Design review of the part shown in the three views and the two pictorial views. Dimensions are in mm from the part's minimum x, y and z. A direction names the side the tool comes from. Give positions to 0.01 mm unless a question says otherwise; leave off trailing zeros. Write each loop counter-clockwise with the first axis right and the second up, starting at its lowest first coordinate (ties: lowest second). Pieces come first, ordered by that corner, then holes. Notation, with made-up numbers: M 39.25,87.5 L 85.25,87.5 A23 ccw 85.25,101.5 Z; hole C -12.5,76.5 d2. An arc over 180 degrees is marked long. Write item = value, one per line.
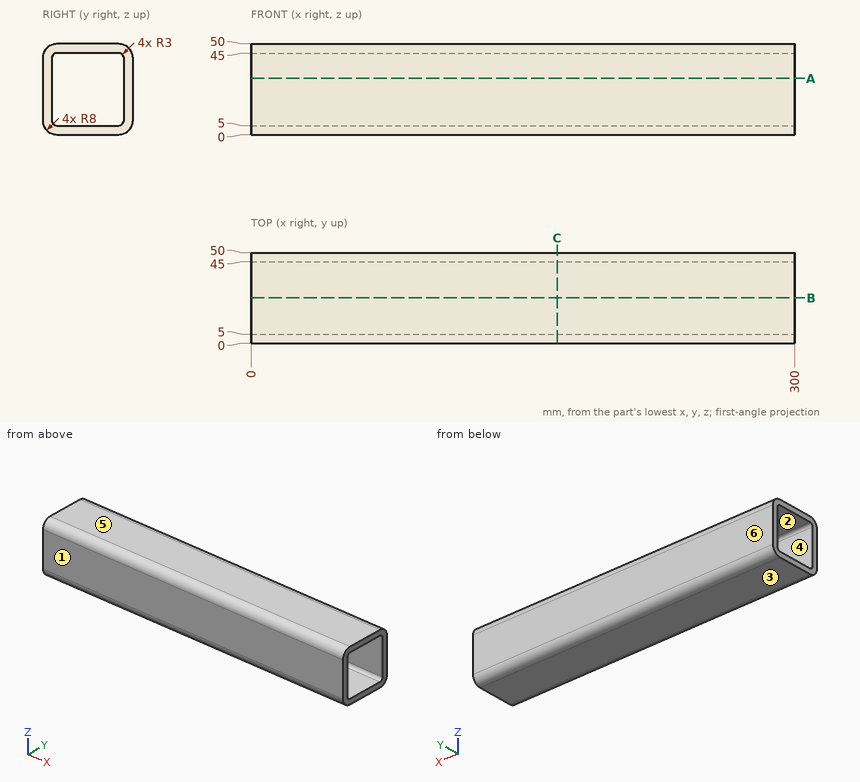
1. The part is to be moulded in two halves that separate along Z. For the marked faces 3, 4, 5 and 6, say which applies: +Z half, -Z half, draft (parallel to the pull), parting line (faces both ways), or undercut.
Responses:
face_3 = -Z half
face_4 = undercut
face_5 = +Z half
face_6 = draft
2. Insertion check: P1, Ø10, axis at y = 14, z = 39.5, coming from the -X side; P2, Ø4, axis at x = 216, y = 5.5, coming from the -Z side. Each pin has a flat end and moves straight along its axis. Give the tip position at first contact, or say it passes through.
Responses:
P1 = through
P2 = 0.02
3. We need section A-A, the plane z = 31. Write out the cut boundary in (x, y).
Responses:
outline = M 0,0 L 300,0 L 300,5 L 0,5 Z; M 0,45 L 300,45 L 300,50 L 0,50 Z
4. Machinability: for the marked faces 1 and 2, which of the approach directions +Z, -Z, +X, -X, +Y, -Y give a long, thin tool a straight path to every point of the face, cutting with its end or side? Answer none if there is none.
Responses:
face_1 = +Z, -Z, +X, -X, -Y
face_2 = +X, -X
5. We need section C-C, the plane x = 169. Write out the cut boundary in (y, z), then the cut area to 3 significant figures.
Responses:
outline = M 0,8 A8 ccw 8,0 L 42,0 A8 ccw 50,8 L 50,42 A8 ccw 42,50 L 8,50 A8 ccw 0,42 Z; hole M 5,8 A3 ccw 8,5 L 42,5 A3 ccw 45,8 L 45,42 A3 ccw 42,45 L 8,45 A3 ccw 5,42 Z
area = 853 mm2
6. For line 1 along Y through (x, z) = (142, 20.5); line 2 along Z through (x, y) = (264, 3) (3 decimals), list the stretches that pass through material, from the lowest coordinate up. Write a range as from..to.
Responses:
line_1 = 0..5, 45..50
line_2 = 1.755..48.245
